from build123d import *

# Parameters (mm, degrees)
SKETCH_1_W              = 150
SKETCH_1_H              = 260
EXTRUDE_1_DEPTH         = 12
FILLET_1_R              = 6
HOLE_WIZARD_M20_1_D     = 17.5
HOLE_WIZARD_M20_1_DEPTH = 47.5
HOLE_WIZARD_M20_1_TIP   = 5.257530416
HOLE_WIZARD_M10_1_D     = 8.5
HOLE_WIZARD_M10_1_DEPTH = 24.5
HOLE_WIZARD_M10_1_TIP   = 2.553657631


with BuildPart() as part:
    # 草图1 → 凸台-拉伸1 (new body)
    with BuildSketch(Plane(origin=(0, 0, 0), x_dir=(1, 0, 0), z_dir=(0, 1, 0))):
        Rectangle(SKETCH_1_W, SKETCH_1_H)
    extrude(amount=EXTRUDE_1_DEPTH)

    # 圆角1
    fillet_1_edges = [part.edges().sort_by_distance(p)[0] for p in [
        (75, 6, 130),
        (-75, 6, 130),
        (-75, 6, -130),
        (75, 6, -130),
    ]]
    fillet(fillet_1_edges, radius=FILLET_1_R)

    # M20 螺纹孔1
    with Locations(Plane(origin=(0, 0, 0), x_dir=(-1, 0, 0), z_dir=(0, -1, 0))):
        with Locations((0, 60)):
            Hole(HOLE_WIZARD_M20_1_D / 2, depth=HOLE_WIZARD_M20_1_DEPTH)
            with Locations((0, 0, -(HOLE_WIZARD_M20_1_DEPTH + HOLE_WIZARD_M20_1_TIP / 2))):  # 118° drill point
                Cone(0, HOLE_WIZARD_M20_1_D / 2, HOLE_WIZARD_M20_1_TIP, mode=Mode.SUBTRACT)

    # M10 螺纹孔1
    with Locations(Plane(origin=(0, 0, 0), x_dir=(-1, 0, 0), z_dir=(0, -1, 0))):
        with Locations((62.5, -117.5), (62.5, -42.5), (-12.5, -42.5), (-12.5, -117.5)):
            Hole(HOLE_WIZARD_M10_1_D / 2, depth=HOLE_WIZARD_M10_1_DEPTH)
            with Locations((0, 0, -(HOLE_WIZARD_M10_1_DEPTH + HOLE_WIZARD_M10_1_TIP / 2))):  # 118° drill point
                Cone(0, HOLE_WIZARD_M10_1_D / 2, HOLE_WIZARD_M10_1_TIP, mode=Mode.SUBTRACT)


solid = part.part
Here's how the part is built. I have some questions about the finished solid (model axes, mm). Round coordinates to 2 decimals unless told otherwise and drop trailing zeros. Order: outer loops, then holes, each group sorted by start corner. A loop starts at its lowest first (then second) coordinate and runs counter-clockwise, first axis right, second up. Notation, with made-up numbers: M -23.5,58.25 L -13.5,58.25 A21 cw -13.5,69.25 Z; hole C -6,-10 d3. An arc over 180 degrees is marked long. Return JSON: item names as keys, results as strings. Group by question number.
1. Please list where these lines run through material, in increasing order: probe 1 along X at (y, z) = (8.5, 42.5); probe 2 along Z at (x, y) = (-62.5, 3.5); probe 3 along Z at (x, y) = (0, 6.75).
2. If we section it at D-D on z = 117.5: List the corners of the cut face in (x, y) for me, then the cut area to 3 significant figures.
3. If we section it at C-C on x = 0: List the corners of the cut face in (y, z) for me.
4. I'm going to push a flat-ended pin straight in: pin 1 Ø7.5 at (x, z) = (-62.5, 117.5) entering from +Y. Where does the tip first touch, or does it pass through?
5. If we section it at A-A on z = -60: List the corners of the cut face in (x, y) for me.
6. If we mould it in two halves opening along X, with no side actions, what happens to faces 1 (the face through (-1.139, 6.084, -68.676)), 2 (the face through (73.289, 6.084, -128.196)), 3 (the face through (-75, 6, 2))? For each: pulls with the +X half, pulls with the -X half, needs draft (parallel to the pull), parting line crosses it, or undercut.
7. If we section it at B-B on x = -62.5: List the corners of the cut face in (y, z) for me, then the cut area to 3 significant figures.
Reply:
{
 "1": {"probe 1": "-75 to -66.75, -58.25 to 8.25, 16.75 to 75", "probe 2": "-130 to 38.25, 46.75 to 113.25, 121.75 to 130", "probe 3": "-130 to -68.75, -51.25 to 130"},
 "2": {"outline": "M -75,0 L -66.75,0 L -66.75,12 L -75,12 Z; M -58.25,0 L 8.25,0 L 8.25,12 L -58.25,12 Z; M 16.75,0 L 75,0 L 75,12 L 16.75,12 Z", "area": "1,600 mm^2"},
 "3": {"outline": "M 0,-130 L 12,-130 L 12,-68.75 L 0,-68.75 Z; M 0,-51.25 L 12,-51.25 L 12,130 L 0,130 Z"},
 "4": {"pin 1": "through"},
 "5": {"outline": "M -75,0 L -8.75,0 L -8.75,12 L -75,12 Z; M 8.75,0 L 75,0 L 75,12 L 8.75,12 Z"},
 "6": {"face 1": "undercut", "face 2": "pulls with the +X half", "face 3": "pulls with the -X half"},
 "7": {"outline": "M 0,-130 L 12,-130 L 12,38.25 L 0,38.25 Z; M 0,46.75 L 12,46.75 L 12,113.25 L 0,113.25 Z; M 0,121.75 L 12,121.75 L 12,130 L 0,130 Z", "area": "2,920 mm^2"}
}
